Answer from the drawing. Dimensions are ordinates in mm from the lowest x, y and z of the part. A direction names the side the tool comes from. Give positions to 0.01 mm unless a question says otherwise; leave off trailing zeros. Loops run counter-clockwise (first coordinate to the right, second up) from the corner with the lowest first, then second, coordinate; pieces in that order, holes last. Notation, with made-up numbers: (62, -37.5) - (77, -37.5) arc R25 ccw to (77, -23.5) - close; hole circle Ø1 at (46, 63.25). An arc over 180 degrees is marked (long way). Answer as CSV lines item,"result". Start each with the question number.
1) For a pull along X with two mould halves and no side action, classify the marked faces 1, 2, 3 and 4 as pulls with the +X half, pulls with the -X half, needs draft (parallel to the pull), parting line crosses it, or undercut.
2) For the marked faces 5 and 6, determine the directions among +Z, -Z, +X, -X, +Y, -Y from which every point of the face is accessible in a straight line to the end or side of a thin tool.
3) A cutting plane is placed at C-C (z = 71). Determine the outline of the cut face in (x, y), and give its area (3 significant figures).
4) A cutting plane is placed at B-B (y = 10.5). Determine the outline of the cut face in (x, z), and give its area (3 significant figures).
5) A flat-ended cylindrical pin translates along its axis: pin 1 (1.5 mm diameter, centred on x = 129, z = 85, fed in from -Y). Find the tip coordinate at first contact, or state that the pin passes through.
6) A cutting plane is placed at A-A (x = 95). Determine the outline of the cut face in (y, z).
7) Find the intervals of material crossed by line 1 along Z through (x, y) = (136.5, 37); line 2 along X through (y, z) = (10, 64); line 3 along Y through (x, z) = (136.5, 19.5), in increasing order.
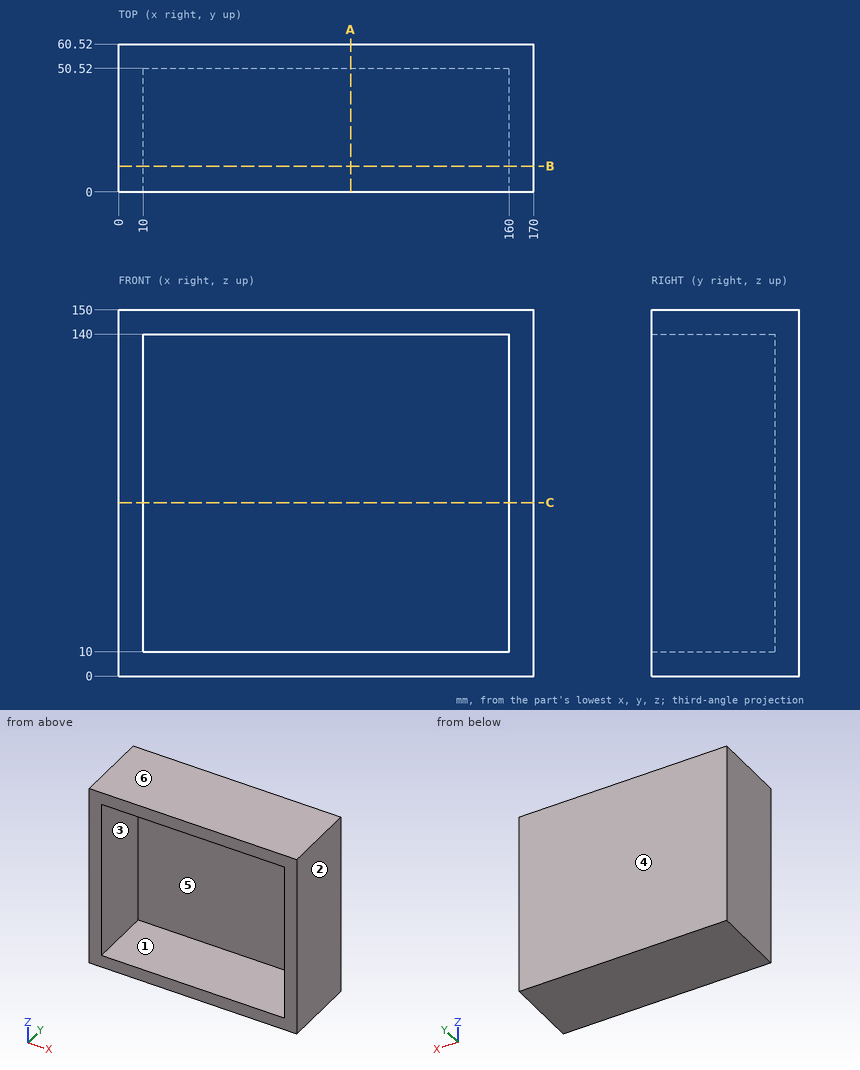
Ans:
1,face 1,"undercut"
1,face 2,"pulls with the +X half"
1,face 3,"undercut"
1,face 4,"needs draft"
2,face 5,"-Y"
2,face 6,"+Z, +X, -X, +Y, -Y"
3,outline,"(0, 0) - (10, 0) - (10, 50.52) - (160, 50.52) - (160, 0) - (170, 0) - (170, 60.52) - (0, 60.52) - close"
3,area,"2,710 mm2"
4,outline,"(0, 0) - (170, 0) - (170, 150) - (0, 150) - close; hole (10, 10) - (160, 10) - (160, 140) - (10, 140) - close"
4,area,"6,000 mm2"
5,pin 1,"y = 50.52"
6,outline,"(0, 0) - (60.52, 0) - (60.52, 150) - (0, 150) - (0, 140) - (50.52, 140) - (50.52, 10) - (0, 10) - close"
7,line 1,"0 to 10, 140 to 150"
7,line 2,"0 to 10, 160 to 170"
7,line 3,"50.52 to 60.52"
